Read the model definition and answer for the solid it produces. Units are mm, in the model's axes. Coordinates: 2 decimals unless noted, no trailing zeros. Loops run counter-clockwise (first coordinate to the right, second up) from the corner with the lowest first, then second, coordinate; pieces in that order, holes last. Notation, with made-up numbers: (-23.5, 4) -> (21.5, 4) arc R10 cw to (21.5, 22) -> close; hole circle Ø2 at (60, -8.75). An arc over 180 degrees is marked (long way). Answer as a JSON object with one key per item and string values. Group by question number.
Q1. The part is cut by section A-A on y = -150. Write down the section's boundary in (x, z).
Q2. The part is cut by section B-B on z = -19.5. Write down the section's boundary in (x, y).
Q3. The part is cut by section C-C on x = -35. Write down the section's boundary in (y, z), and give its area (3 significant figures).
Q4. Straight lines are drawn through the part: line 1 along Y through (x, z) = (-35, -19.5); line 2 along X through (y, z) = (-142.5, -22). For each, find the intervals that lie inside material, in ascending order. Write a range as [from, to].
Q5. Each of these flat-tipped pins is pushed along its axis until it touches: P1, Ø14.5, axis at x = -35, y = -150, coming from the -Z side; P2, Ø7, axis at x = 35, y = -150, coming from the -Z side. Where does it stop, or does it pass through?
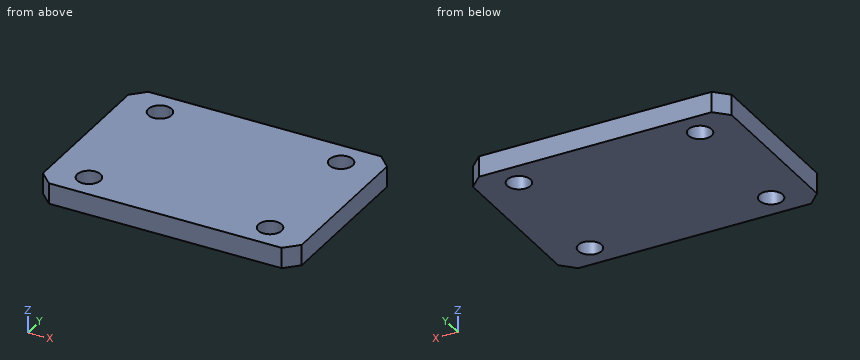
from build123d import *

# Parameters (mm, degrees)
SKETCH1_W           = 100
SKETCH1_H           = 70
BOSS_EXTRUDE1_DEPTH = 8
SKETCH2_R           = 4.5
CUT_EXTRUDE1_DEPTH  = 8
CHAMFER1_SIZE       = 5


with BuildPart() as part:
    # Sketch1 → Boss-Extrude1 (new body)
    with BuildSketch(Plane.XY.offset(-15)):
        with Locations((0, -175)):
            Rectangle(SKETCH1_W, SKETCH1_H)
    extrude(amount=-BOSS_EXTRUDE1_DEPTH)

    # Sketch2 → Cut-Extrude1 (cut)
    with BuildSketch(Plane(origin=(0, 0, -23), x_dir=(-1, 0, 0), z_dir=(0, 0, -1))):
        with Locations((-35, -150)):
            Circle(SKETCH2_R)
        with Locations((35, -150)):
            Circle(SKETCH2_R)
        with Locations((35, -200)):
            Circle(SKETCH2_R)
        with Locations((-35, -200)):
            Circle(SKETCH2_R)
    extrude(amount=-CUT_EXTRUDE1_DEPTH, mode=Mode.SUBTRACT)

    # Chamfer1
    chamfer1_edges = [part.edges().sort_by_distance(p)[0] for p in [
        (50, -210, -19),
        (-50, -210, -19),
        (-50, -140, -19),
        (50, -140, -19),
    ]]
    chamfer(chamfer1_edges, length=CHAMFER1_SIZE)


solid = part.part
Final values:
{
 "1": {"outline": "(-50, -23) -> (-39.5, -23) -> (-39.5, -15) -> (-50, -15) -> close; (-30.5, -23) -> (30.5, -23) -> (30.5, -15) -> (-30.5, -15) -> close; (39.5, -23) -> (50, -23) -> (50, -15) -> (39.5, -15) -> close"},
 "2": {"outline": "(-50, -205) -> (-45, -210) -> (45, -210) -> (50, -205) -> (50, -145) -> (45, -140) -> (-45, -140) -> (-50, -145) -> close; hole circle Ø9 at (-35, -200); hole circle Ø9 at (-35, -150); hole circle Ø9 at (35, -200); hole circle Ø9 at (35, -150)"},
 "3": {"outline": "(-210, -23) -> (-204.5, -23) -> (-204.5, -15) -> (-210, -15) -> close; (-195.5, -23) -> (-154.5, -23) -> (-154.5, -15) -> (-195.5, -15) -> close; (-145.5, -23) -> (-140, -23) -> (-140, -15) -> (-145.5, -15) -> close", "area": "416 mm2"},
 "4": {"line 1": "y = [-210, -204.5], [-195.5, -154.5], [-145.5, -140]", "line 2": "x = [-47.5, 47.5]"},
 "5": {"P1": "stops at z = -23", "P2": "passes through"}
}
